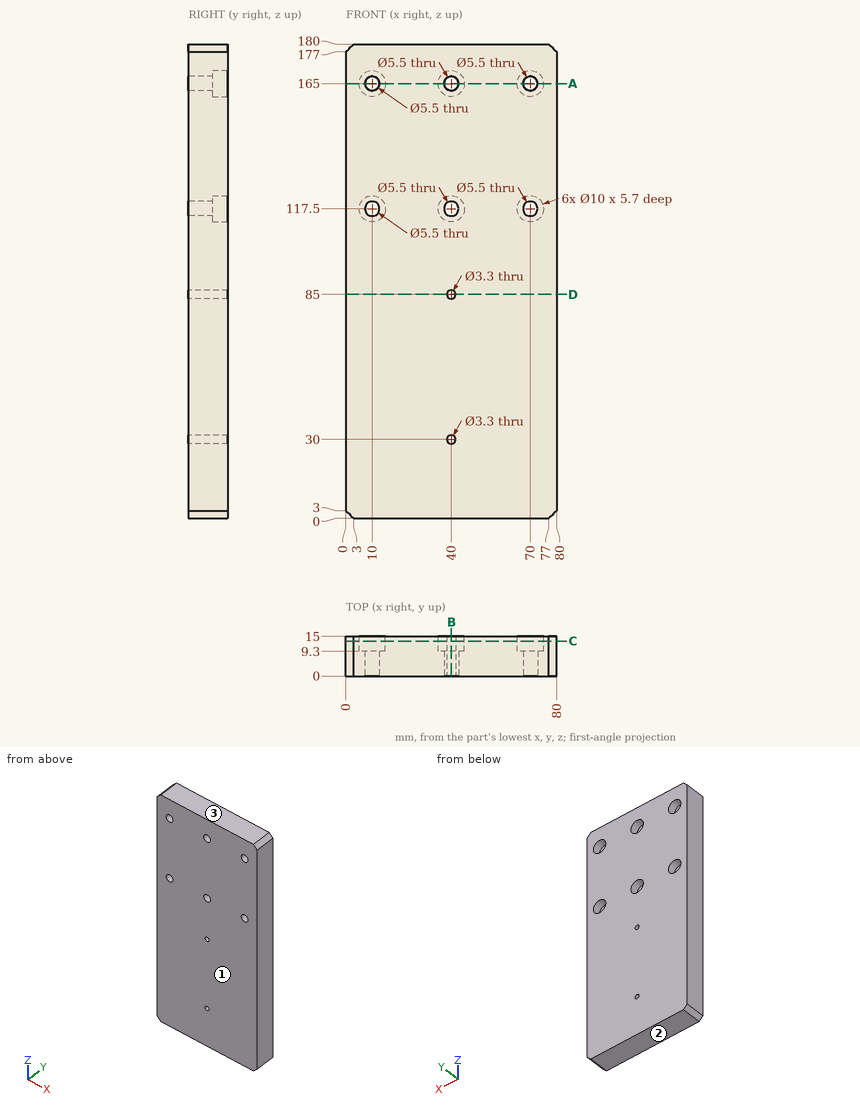
Here's the drawing with two shaded views (mm, measured from the low corner). I have some questions. Coordinates: 2 decimals unless noted, no trailing zeros. Loops run counter-clockwise (first coordinate to the right, second up) from the corner with the lowest first, then second, coordinate; pieces in that order, holes last. Notation, with made-up numbers: (17, 75.5) - (49, 75.5) arc R27 cw to (49, 91.5) - close; hole circle Ø2 at (51.5, 70). An arc over 180 degrees is marked (long way). Answer as CSV lines item,"result". Start each with the question number.
1) Suppose I cut it at A-A (z = 165). Please give me the cut outline in (x, y), plus the area to 3 significant figures.
2) For pin 1 (2 mm diameter, centred on x = 40, z = 85, fed in from -Y); pin 2 (6.5 mm diameter, centred on x = 40, z = 117.5, fed in from +Y); pin 3 (6 mm diameter, centred on y = 4, z = 41.5, fed in from -X), each with a flat end and sliding along its axis, tell me the tip position at first contact or that it passes through.
3) Suppose I cut it at C-C (y = 13.25). Count the separate pieces of the cut face and the enclosed holes in it, plus the area to 3 significant figures.
4) Thinking about a two-plate mould opening in Z: for the marked faces 1, 2 and 3, which applies, pulls with the +Z half, pulls with the -Z half, needs draft (parallel to the pull), parting line crosses it, or undercut?
5) Suppose I cut it at D-D (z = 85). Please give me the cut outline in (x, y).
6) I need wall thicknesses on line 1 (X direction, y = 3.25, z = 165); line 2 (Z direction, x = 40, y = 10.25); line 3 (Z direction, x = 70, y = 13.3). Which ranges of each line are inside material? Lowest first, please. Write a range as from..to.
7) Suppose I cut it at B-B (x = 40). Please give me the cut outline in (y, z), plus the area to 3 significant figures.
Check result:
1,outline,"(0, 0) - (7.25, 0) - (7.25, 9.3) - (5, 9.3) - (5, 15) - (0, 15) - close; (12.75, 0) - (37.25, 0) - (37.25, 9.3) - (35, 9.3) - (35, 15) - (15, 15) - (15, 9.3) - (12.75, 9.3) - close; (42.75, 0) - (67.25, 0) - (67.25, 9.3) - (65, 9.3) - (65, 15) - (45, 15) - (45, 9.3) - (42.75, 9.3) - close; (72.75, 0) - (80, 0) - (80, 15) - (75, 15) - (75, 9.3) - (72.75, 9.3) - close"
1,area,"876 mm²"
2,pin 1,"passes through"
2,pin 2,"stops at y = 9.3"
2,pin 3,"stops at x = 0"
3,separate pieces,"1"
3,enclosed holes,"8"
3,area,"13,900 mm²"
4,face 1,"needs draft"
4,face 2,"pulls with the -Z half"
4,face 3,"pulls with the +Z half"
5,outline,"(0, 0) - (38.35, 0) - (38.35, 15) - (0, 15) - close; (41.65, 0) - (80, 0) - (80, 15) - (41.65, 15) - close"
6,line 1,"x = 0..7.25, 12.75..37.25, 42.75..67.25, 72.75..80"
6,line 2,"z = 0..28.35, 31.65..83.35, 86.65..112.5, 122.5..160, 170..180"
6,line 3,"z = 0..112.5, 122.5..160, 170..180"
7,outline,"(0, 0) - (15, 0) - (15, 28.35) - (0, 28.35) - close; (0, 31.65) - (15, 31.65) - (15, 83.35) - (0, 83.35) - close; (0, 86.65) - (15, 86.65) - (15, 112.5) - (9.3, 112.5) - (9.3, 114.75) - (0, 114.75) - close; (0, 120.25) - (9.3, 120.25) - (9.3, 122.5) - (15, 122.5) - (15, 160) - (9.3, 160) - (9.3, 162.25) - (0, 162.25) - close; (0, 167.75) - (9.3, 167.75) - (9.3, 170) - (15, 170) - (15, 180) - (0, 180) - close"
7,area,"2,380 mm²"
